Geometry: final body of the model. Coordinates: model frame, mm. A direction names the side the tool comes from. Give positions to 0.01 mm unless a question says otherwise; leave off trailing zeros. Order: outer loops, then holes, each group sorted by start corner. A loop starts at its lowest first (then second) coordinate and runs counter-clockwise, first axis right, second up. Notation, with made-up numbers: (68.25, -6) - (127.25, -6) arc R19 cw to (127.25, 12) - close; hole circle Ø1 at (47, 25.25). An arc over 180 degrees is marked (long way). Put each result on its own line as item: value. Start each with the question number.
1. Ray query, line 1 along Y through (x, z) = (33.5, 23); line 2 along Y through (x, z) = (34, 24); line 3 along Z through (x, y) = (18.5, 22). Return the intervals inside material, ascending. Write a range as from..to.
2. Section D-D on y = 21. Return the cut outline in (x, z).
3. Section C-C on y = 12.5. Return the cut outline in (x, z), plus the area to 3 significant figures.
4. Set-up query: faces 5 (the flat face through (7.4, 32.1, 3)), 6 (the flat face through (29, 22, 23)), 7 (the flat face through (21, 23, 6)). Return all of +Z, -Z, +X, -X, +Y, -Y with unobstructed straight access to the full face (end or side cutting, diameter ignored); none if empty.
5. First-contact query: P1, Ø19, axis at y = 12.5, z = 23, coming from the -X side; P2, Ø5.5, axis at x = 31, y = 22, coming from the +Z side; P3, Ø10, axis at x = 21, y = 11.5, coming from the +Z side. Flat tips, straight axial feed; report the tip coordinate or a pass-through.
6. Section A-A on z = 23. Return the cut outline in (x, y), plus the area to 3 significant figures.
7. Mould query, pull axis Z, two halves, no side actions, for faces 1 (the flat face through (24, 23, 0)), 2 (the flat face through (17, 22, 3)), 3 (the flat face through (31, 22, 35)), 4 (the flat face through (31, 22, 11)). Classes: pulls with the +Z half, pulls with the -Z half, needs draft (parallel to the pull), parting line crosses it, or undercut.
8. Section B-B on x = 12. Return the cut outline in (y, z).
from build123d import *

# Parameters (mm, degrees)
BASE_PLATE_SKETCH_W        = 40
BASE_PLATE_SKETCH_H        = 45
BASE_PLATE_DEPTH           = 6
UPRIGHT_FLANGE_SKETCH_W    = 34
UPRIGHT_FLANGE_SKETCH_H    = 45
UPRIGHT_FLANGE_DEPTH       = 6
SUPPORT_WEB_SKETCH_W       = 5
SUPPORT_WEB_SKETCH_H       = 24
SUPPORT_WEB_DEPTH          = 45
CORNER_RELIEF_GROOVE_DEPTH = 45
MOUNTING_HOLES_SKETCH_R    = 6
MOUNTING_HOLES_2X_DEPTH    = 45


with BuildPart() as part:
    # Base Plate Sketch → Base Plate (new body)
    with BuildSketch(Plane.XY):
        with Locations((20, 22.5)):
            Rectangle(BASE_PLATE_SKETCH_W, BASE_PLATE_SKETCH_H)
    extrude(amount=BASE_PLATE_DEPTH)

    # Upright Flange Sketch → Upright Flange (add)
    with BuildSketch(Plane(origin=(40, 0, 0), x_dir=(0, 0, -1), z_dir=(1, 0, 0))):
        with Locations((-23, 22.5)):
            Rectangle(UPRIGHT_FLANGE_SKETCH_W, UPRIGHT_FLANGE_SKETCH_H)
    extrude(amount=-UPRIGHT_FLANGE_DEPTH)

    # Support Web Sketch → Support Web (add)
    with BuildSketch(Plane.XZ):
        with Locations((31.5, 23)):
            Rectangle(SUPPORT_WEB_SKETCH_W, SUPPORT_WEB_SKETCH_H)
    extrude(amount=-SUPPORT_WEB_DEPTH)

    # Corner Relief Groove Sketch → Corner Relief Groove (cut)
    with BuildSketch(Plane.XY.offset(6)):
        Polygon((0, 39.5), (0, 22.5), (17, 22.5), (17, 25), (14.5, 25), align=None)
        Polygon((17, 22.5), (0, 22.5), (0, 5.5), (14.5, 20), (17, 20), align=None)
    extrude(amount=-CORNER_RELIEF_GROOVE_DEPTH, mode=Mode.SUBTRACT)

    # Mounting Holes Sketch → Mounting Holes 2x (cut)
    with BuildSketch(Plane.ZY.offset(-29)):
        with Locations((23, 32.5)):
            Circle(MOUNTING_HOLES_SKETCH_R)
        with Locations((23, 12.5)):
            Circle(MOUNTING_HOLES_SKETCH_R)
    extrude(amount=-MOUNTING_HOLES_2X_DEPTH, mode=Mode.SUBTRACT)


solid = part.part
Resolved:
1. line 1: 0..6.5, 18.5..26.5, 38.5..45
1. line 2: 0..6.58, 18.42..26.58, 38.42..45
1. line 3: 0..6
2. outline: (17, 0) - (40, 0) - (40, 40) - (34, 40) - (34, 35) - (29, 35) - (29, 11) - (34, 11) - (34, 6) - (17, 6) - close
3. outline: (7, 0) - (40, 0) - (40, 17) - (29, 17) - (29, 11) - (34, 11) - (34, 6) - (7, 6) - close; (29, 29) - (40, 29) - (40, 40) - (34, 40) - (34, 35) - (29, 35) - close
3. area: 390 mm^2
4. face 5: +Z, -Z, -X
4. face 6: +Z, -X, +Y, -Y
4. face 7: -X, +Y, -Y
5. P1: x = 29
5. P2: z = 35
5. P3: z = 6
6. outline: (29, 0) - (40, 0) - (40, 6.5) - (29, 6.5) - close; (29, 18.5) - (40, 18.5) - (40, 26.5) - (29, 26.5) - close; (29, 38.5) - (40, 38.5) - (40, 45) - (29, 45) - close
6. area: 231 mm^2
7. face 1: pulls with the -Z half
7. face 2: needs draft
7. face 3: pulls with the +Z half
7. face 4: undercut
8. outline: (0, 0) - (17.5, 0) - (17.5, 6) - (0, 6) - close; (27.5, 0) - (45, 0) - (45, 6) - (27.5, 6) - close
